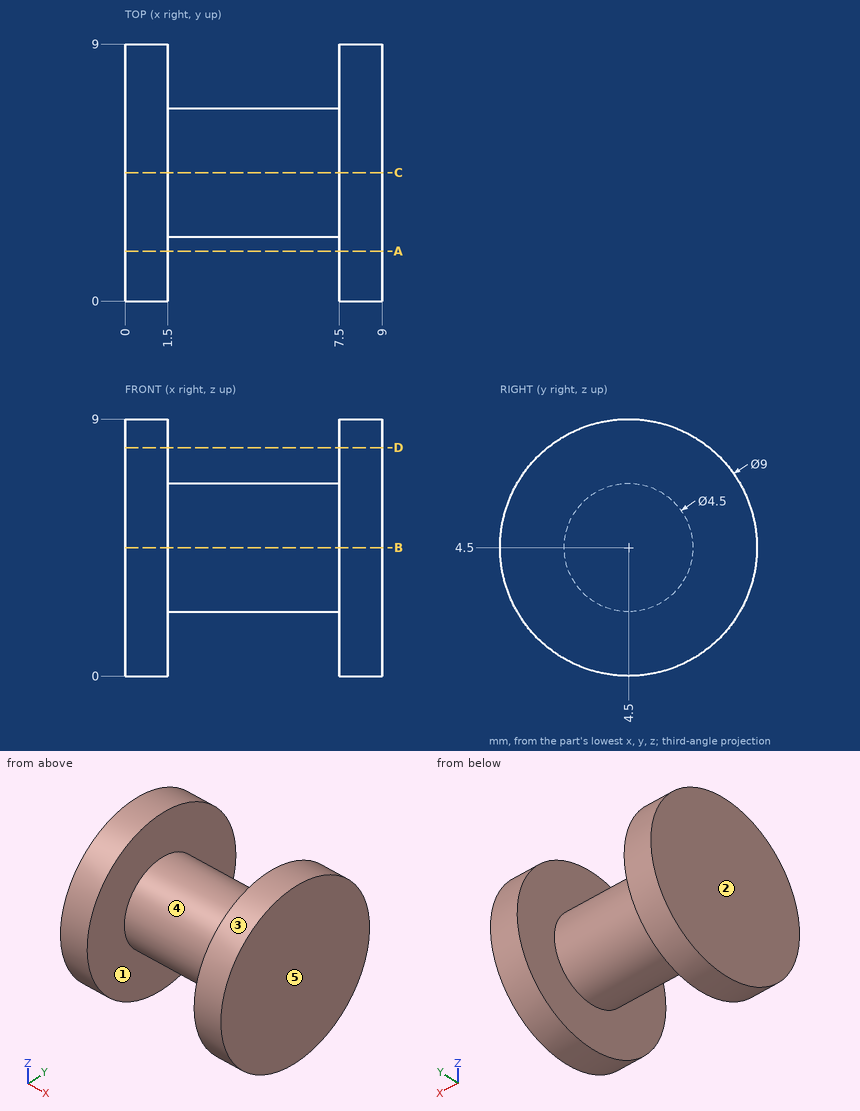
Design review of the part shown in the three views and the two pictorial views. Dimensions are in mm from the part's minimum x, y and z. A direction names the side the tool comes from. Coordinates: 2 decimals unless noted, no trailing zeros. Order: outer loops, then holes, each group sorted by start corner. A loop starts at its lowest first (then second) coordinate and runs counter-clockwise, first axis right, second up. Notation, with made-up numbers: (-22, 60.25) - (-12, 60.25) arc R20 ccw to (-12, 87.25) - close; hole circle Ø2 at (10, -40). An arc over 180 degrees is marked (long way). Answer as CSV lines item,"result". Start each with the question number.
1) Machinability: for the marked faces 4 and 5, which of the approach directions +Z, -Z, +X, -X, +Y, -Y give a long, thin tool a straight path to every point of the face, cutting with its end or side? Answer none if there is none.
2) Add section D-D (z = 8). State the section outline as (x, y) points, then the cut area to 3 significant figures.
3) To check wall thickness, follow line 1 along X through (y, z) = (3.25, 8.5); line 2 along Y through (x, z) = (5.5, 4.5); line 3 along Z through (x, y) = (1, 6.5). State the ranges of each line that lie inside material, in increasing order. Write a range as [from, to].
4) Add section A-A (y = 1.75). State the section outline as (x, z) points, then the cut area to 3 significant figures.
5) Insertion check: P1, Ø3, axis at x = 6.5, y = 6.5, coming from the +Z side; P2, Ø4, axis at x = 2.5, z = 2.5, coming from the -Y side; P3, Ø1, axis at x = 8, y = 3.5, coming from the +Z side. Each pin has a flat end and moves straight along its axis. Give the tip position at first contact, or say it passes through.
6) Draft analysis for pull direction X (two halves, no side actions). For the marked faces 1, 2 and 3, state which applies: +X half, -X half, draft (parallel to the pull), parting line (faces both ways), or undercut.
7) Add section B-B (z = 4.5). State the section outline as (x, y) points.
Result:
1,face 4,"none"
1,face 5,"+Z, -Z, +X, +Y, -Y"
2,outline,"(0, 1.67) - (1.5, 1.67) - (1.5, 7.33) - (0, 7.33) - close; (7.5, 1.67) - (9, 1.67) - (9, 7.33) - (7.5, 7.33) - close"
2,area,"17.0 mm^2"
3,line 1,"[0, 1.5], [7.5, 9]"
3,line 2,"[2.25, 6.75]"
3,line 3,"[0.47, 8.53]"
4,outline,"(0, 0.94) - (1.5, 0.94) - (1.5, 8.06) - (0, 8.06) - close; (7.5, 0.94) - (9, 0.94) - (9, 8.06) - (7.5, 8.06) - close"
4,area,"21.4 mm^2"
5,P1,"z = 8.91"
5,P2,"y = 0.01"
5,P3,"z = 8.97"
6,face 1,"undercut"
6,face 2,"-X half"
6,face 3,"draft"
7,outline,"(0, 0) - (1.5, 0) - (1.5, 2.25) - (7.5, 2.25) - (7.5, 0) - (9, 0) - (9, 9) - (7.5, 9) - (7.5, 6.75) - (1.5, 6.75) - (1.5, 9) - (0, 9) - close"
